Geometry check sheet. Reference: the model listing, model coordinates, mm. Face numbers are marked on the shaded views. A direction names the side the tool comes from. Round coordinates to 2 decimals unless told otherwise and drop trailing zeros. Order: outer loops, then holes, each group sorted by start corner. A loop starts at its lowest first (then second) coordinate and runs counter-clockwise, first axis right, second up.
(1) Set-up check for the marked faces 4, 5, 6 and 7: record each of +Z, -Z, +X, -X, +Y, -Y from which the full face is reachable in a straight line by a thin tool's end or side.
(2) Sectioned sample at C-C (x = -1.5). Record the boundary of the cut face in (y, z), plus the area to 3 significant figures.
(3) Sectioned sample at A-A (x = 9). Record the boundary of the cut face in (y, z).
(4) Go/stop test with flat-tipped pins: pin 1 (9.5 mm diameter, centred on y = 33.58, z = -107.66, fed in from -X); pin 2 (6.5 mm diameter, centred on x = 0, z = -65, fed in from +Y); pin 3 (8 mm diameter, centred on x = -2.5, z = -70.5, fed in from -Y); pin 4 (3 mm diameter, centred on x = -6, z = -65, fed in from +Y). Record where each tip stops, or that it passes through.
(5) Material ranges on line 1 along X through (y, z) = (32, -20); line 2 along X through (y, z) = (55.25, -65); line 3 along Y through (x, z) = (14, -9), recorded low to high.
(6) Sectioned sample at B-B (z = -65). Record the boundary of the cut face in (x, y), plus the area to 3 significant figures.
(7) Sectioned sample at D-D (y = 43.5). Record the boundary of the cut face in (x, z).
(8) Release check for a two-part mould opening along Z. For the marked faces 1, 2 and 3 record: +Z half, -Z half, draft (parallel to the pull), parting line (faces both ways), or undercut.
from build123d import *

# Parameters (mm, degrees)
HOUSING_BODY_DEPTH       = 20
CORNER_CUT_A_6X6_DEPTH   = 101.816665289
CORNER_CUT_B_6X6_DEPTH   = 101.816665289
STEP_HOLE_SKETCH_R       = 6
STEP_HOLE_CUT_DEPTH      = 11
SECOND_STEP_CUT_SKETCH_R = 5.5
SECOND_STEP_CUT_DEPTH    = 11
EYE_LUG_DEPTH            = 20
EYE_BORE_SKETCH_R        = 6
EYE_BORE_12_DEPTH        = 147.389505053


with BuildPart() as part:
    # Housing Profile Sketch → Housing Body (new, symmetric)
    with BuildSketch(Plane(origin=(0, 0, 0), x_dir=(0, 0, -1), z_dir=(1, 0, 0))):
        with BuildLine():
            Line((0, 0), (40, 0))
            ThreePointArc((40, 0), (44.522774425, 8.366600265), (54, 9.16515139))
            Line((54, 9.16515139), (80, 9.16515139))
            Line((80, 9.16515139), (80, 58))
            Line((80, 58), (50.341394733, 58))
            Line((50.341394733, 58), (39.949089887, 40))
            Line((39.949089887, 40), (0, 40))
            Line((0, 40), (0, 0))
        make_face()
    extrude(amount=HOUSING_BODY_DEPTH, both=True)

    # Corner Cut A Sketch → Corner Cut A 6x6 (cut, through all)
    with BuildSketch(Plane.XZ):
        Polygon((14, 0), (20, -6), (20, 0), align=None)
    extrude(amount=-CORNER_CUT_A_6X6_DEPTH, mode=Mode.SUBTRACT)

    # Corner Cut B Sketch → Corner Cut B 6x6 (cut, through all)
    with BuildSketch(Plane.XZ):
        Polygon((-20, 0), (-20, -6), (-14, 0), align=None)
    extrude(amount=-CORNER_CUT_B_6X6_DEPTH, mode=Mode.SUBTRACT)

    # Step Hole Sketch → Step Hole Cut (cut)
    with BuildSketch(Plane(origin=(0, 40, 0), x_dir=(1, 0, 0), z_dir=(0, 1, 0))):
        with Locations(Location((0, 20, 0), (0, 0, 270))):
            Circle(STEP_HOLE_SKETCH_R)
    extrude(amount=-STEP_HOLE_CUT_DEPTH, mode=Mode.SUBTRACT)

    # Second Step Cut Sketch → Second Step Cut (cut)
    with BuildSketch(Plane(origin=(0, 58, 0), x_dir=(1, 0, 0), z_dir=(0, 1, 0))):
        with Locations(Location((0, 65, 0), (0, 0, 270))):
            Circle(SECOND_STEP_CUT_SKETCH_R)
    extrude(amount=-SECOND_STEP_CUT_DEPTH, mode=Mode.SUBTRACT)

    # Eye Lug Sketch → Eye Lug (add)
    with BuildSketch(Plane.ZY.offset(20)):
        with BuildLine():
            Line((-107.657336829, 58.582575695), (-80, 58))
            Line((-80, 58), (-80, 9.16515139))
            Line((-80, 9.16515139), (-107.657336829, 8.582575695))
            ThreePointArc((-107.657336829, 8.582575695), (-132.657336829, 33.582575695), (-107.657336829, 58.582575695))
        make_face()
    extrude(amount=-EYE_LUG_DEPTH)

    # Eye Bore Sketch → Eye Bore Ø12 (cut, through all)
    with BuildSketch(Plane(origin=(0, 0, 0), x_dir=(0, 0, -1), z_dir=(1, 0, 0))):
        with Locations((107.657336829, 33.582575695)):
            Circle(EYE_BORE_SKETCH_R)
    extrude(amount=-EYE_BORE_12_DEPTH, mode=Mode.SUBTRACT)


solid = part.part
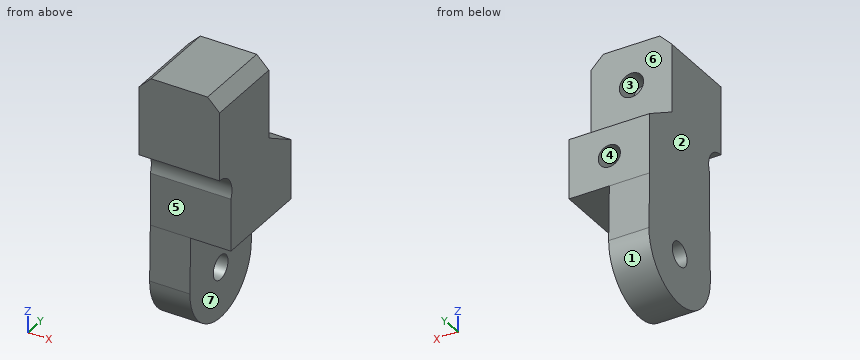
Answer below:
1. face 4: +Y
1. face 5: +X, -X, -Y
1. face 6: +Z, +X, -X, +Y
1. face 7: -Z, +X, +Y, -Y
2. outline: (0, -40) arc R10 cw to (9.17, -54) - (9.17, -80) - (8.58, -107.66) arc R25 ccw to (58.58, -107.66) - (58, -80) - (58, -70.29) - (47, -70.29) - (47, -59.71) - (58, -59.71) - (58, -50.34) - (40, -39.95) - (40, -25.81) - (29, -25.81) - (29, -14.19) - (40, -14.19) - (40, 0) - (0, 0) - close; hole circle Ø12 at (33.58, -107.66)
2. area: 5,460 mm2
3. outline: (0, -40) arc R10 cw to (9.17, -54) - (9.17, -80) - (58, -80) - (58, -50.34) - (40, -39.95) - (40, 0) - (0, 0) - close
4. pin 1: passes through
4. pin 2: stops at y = 47
4. pin 3: stops at y = 9.17
4. pin 4: stops at y = 58
5. line 1: x = -20 to -6, 6 to 20
5. line 2: x = -20 to -5.5, 5.5 to 20
5. line 3: y = 0 to 40
6. outline: (-20, 9.17) - (20, 9.17) - (20, 58) - (5.5, 58) - (5.5, 47) - (-5.5, 47) - (-5.5, 58) - (-20, 58) - close
6. area: 1,830 mm2
7. outline: (-20, -130.61) - (0, -130.61) - (0, -80) - (20, -80) - (20, -41.97) - (-20, -41.97) - close
8. face 1: -Z half
8. face 2: draft
8. face 3: undercut
